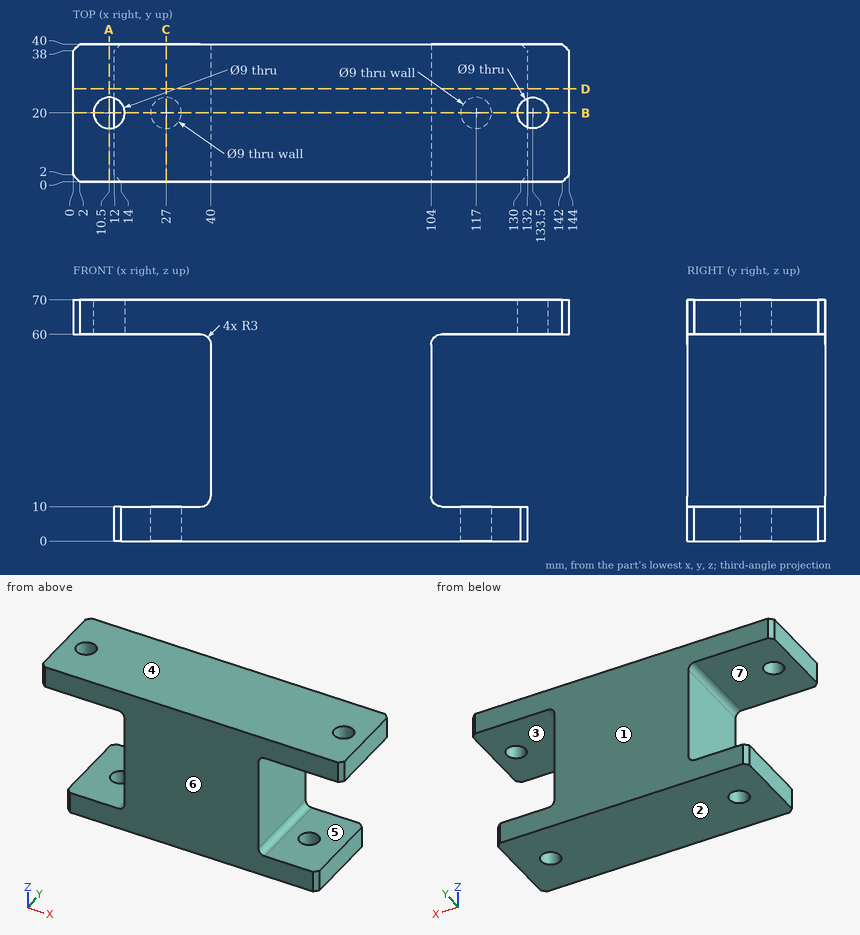
Answer from the drawing. Dimensions are ordinates in mm from the lowest x, y and z of the part. A direction names the side the tool comes from. Give positions to 0.01 mm unless a question says otherwise; leave off trailing zeros. Write each loop counter-clockwise with the first axis right and the second up, starting at its lowest first coordinate (ties: lowest second). Pieces come first, ordered by that corner, then holes.
1) Find the intervals of material crossed by L1, parallel to Z at x = 32, y = 37; L2, parallel to Y at x = 133.5, z = 67; L3, parallel to X at y = 25.5, z = 37.5, in increasing order.
2) Given P1, Ø12, axis at y = 10, z = 34, coming from the +X side; P2, Ø1, axis at y = 11, z = 43, coming from the -X side; P3, Ø3, axis at y = 16.5, z = 5, coming from the -X side, each flat-ended and moving along its own axis, determine where each tip first touches the part or whether it passes through.
3) Section A-A (x = 10.5) is taken. Write down the section's boundary in (y, z).
4) Section C-C (x = 27) is taken. Write down the section's boundary in (y, z).
5) A tool of negligible diameter and unlimited length cuts with its end or side. For the marked faces 5, 6 and 7, from which of +Z, -Z, +X, -X, +Y, -Y can it reach the whole face along a straight path? Write none if from no direction.
6) Section B-B (y = 20) is taken. Count the separate pieces of the cut face and the enclosed holes in it, and give its area (3 significant figures).
7) Section D-D (y = 27) is taken. Write down the section's boundary in (x, z), and give its area (3 significant figures).
8) For a pull along Z with two mould halves and no side action, classify the marked faces 1, 2, 3 and 4 as pulls with the +Z half, pulls with the -Z half, needs draft (parallel to the pull), parting line crosses it, or undercut.
Response:
1. L1: z = 0 to 10, 60 to 70
1. L2: y = 0 to 15.5, 24.5 to 40
1. L3: x = 40 to 104
2. P1: stops at x = 104
2. P2: stops at x = 40
2. P3: stops at x = 12
3. outline: (0, 60) - (15.5, 60) - (15.5, 70) - (0, 70) - close; (24.5, 60) - (40, 60) - (40, 70) - (24.5, 70) - close
4. outline: (0, 0) - (15.5, 0) - (15.5, 10) - (0, 10) - close; (0, 60) - (40, 60) - (40, 70) - (0, 70) - close; (24.5, 0) - (40, 0) - (40, 10) - (24.5, 10) - close
5. face 5: +X, +Y, -Y
5. face 6: +Z, -Z, +X, -X, -Y
5. face 7: -X, +Y, -Y
6. separate pieces: 5
6. enclosed holes: 0
6. area: 5,490 mm2
7. outline: (0, 60) - (37, 60) arc R3 cw to (40, 57) - (40, 13) arc R3 cw to (37, 10) - (12, 10) - (12, 0) - (132, 0) - (132, 10) - (107, 10) arc R3 cw to (104, 13) - (104, 57) arc R3 cw to (107, 60) - (144, 60) - (144, 70) - (0, 70) - close
7. area: 5,850 mm2
8. face 1: needs draft
8. face 2: pulls with the -Z half
8. face 3: undercut
8. face 4: pulls with the +Z half
